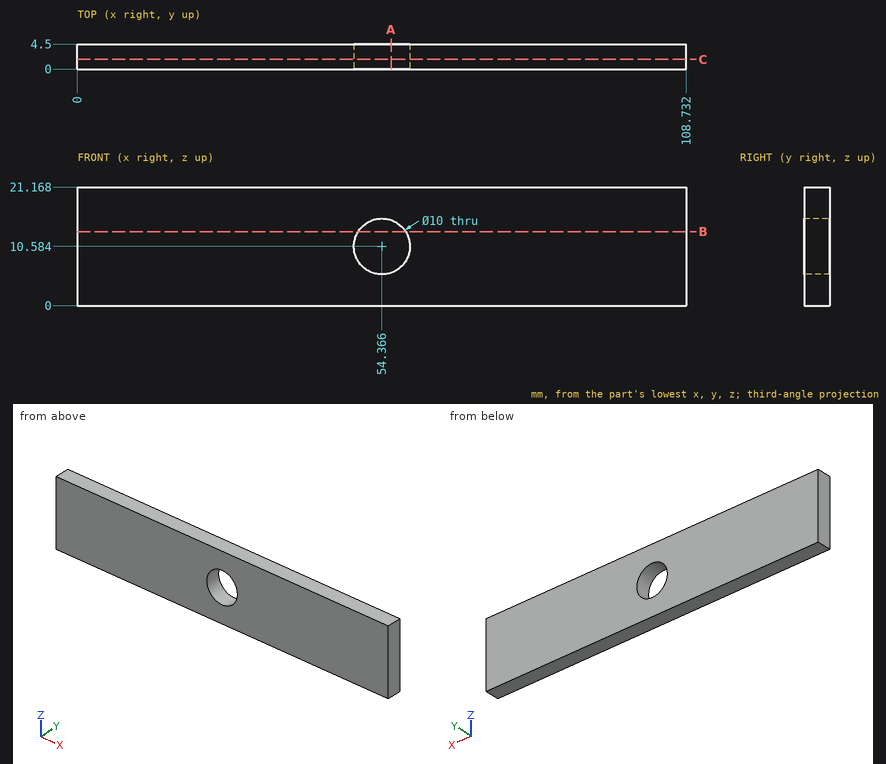
Part print with two shaded views. Sizes in mm from the minimum x, y, z corner. Round coordinates to 2 decimals unless told otherwise and drop trailing zeros. Order: outer loops, then holes, each group sorted by start corner. A loop starts at its lowest first (then second) coordinate and runs counter-clockwise, first axis right, second up. Notation, with made-up numbers: M 72,44.5 L 76,44.5 A11 ccw 76,55.5 Z; hole C 78,50 d7. An arc over 180 degrees is marked long. Put each result on its own line as item: value. Start each with the question number.
1. Slice it at B-B on z = 13.25. List the corners of the cut face in (x, y), then the cut area to 3 significant figures.
2. Drill centre lines: probe 1 along X at (y, z) = (0.3, 9.5) (1 decimal); probe 2 along X at (y, z) = (1.5, 7.75) (1 decimal). Where is each one in solid material? Low to high. Write a range as [from, to].
3. Drop a flat-ended pin along its axis: pin 1 (2 mm diameter, centred on x = 19, y = 2.5, fed in from -Z). Give the stop position or say it passes through.
4. Slice it at A-A on x = 56. List the corners of the cut face in (y, z), then the cut area to 3 significant figures.
5. Slice it at C-C on y = 1.75. List the corners of the cut face in (x, z).
Findings:
1. outline: M 0,0 L 50.14,0 L 50.14,4.5 L 0,4.5 Z; M 58.6,0 L 108.73,0 L 108.73,4.5 L 58.6,4.5 Z
1. area: 451 mm2
2. probe 1: [0, 49.5], [59.2, 108.7]
2. probe 2: [0, 50.2], [58.5, 108.7]
3. pin 1: z = 0
4. outline: M 0,0 L 4.5,0 L 4.5,5.86 L 0,5.86 Z; M 0,15.31 L 4.5,15.31 L 4.5,21.17 L 0,21.17 Z
4. area: 52.7 mm2
5. outline: M 0,0 L 108.73,0 L 108.73,21.17 L 0,21.17 Z; hole C 54.37,10.58 d10
